Input: part model. Units: mm. Frame: model coordinates. Face numbers are marked on the shaded views. A direction names the side the tool comes from. Give positions to 0.01 mm unless a question says otherwise; leave off trailing zeros. Order: outer loops, then holes, each group sorted by start corner. A loop starts at its lowest first (then second) coordinate and runs counter-clockwise, first axis right, second up. Notation, with made-up numbers: (60.5, 57.5) - (101.5, 57.5) arc R13 cw to (101.5, 67.5) - close; hole circle Ø4 at (17, 77). An arc over 180 degrees is marked (long way). Answer in a Markdown table with one row per item. Add a question column.
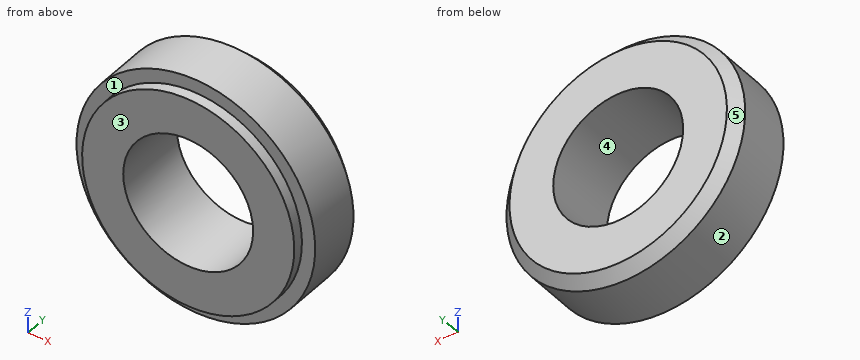
from build123d import *

# Parameters (mm, degrees)
G3_4_TAPPED_HOLE1_D     = 24.5
G3_4_TAPPED_HOLE1_DEPTH = 58.32
G3_4_TAPPED_HOLE1_TIP   = 7.360542583


with BuildPart() as part:
    # Sketch1 → Revolve1 (revolve)
    with BuildSketch(Plane(origin=(0, 0, 0), x_dir=(0, 0, -1), z_dir=(1, 0, 0))):
        Polygon((20, 0), (20, 2), (22.5, 2), (22.5, 12), (20.5, 14), (12, 14), (12, 0), align=None)
    revolve(axis=Axis((0, 0, 0), (0, 1, 0)))

    # G3/4 Tapped Hole1
    with Locations(Plane(origin=(0, 14, 0), x_dir=(1, 0, 0), z_dir=(0, 1, 0))):
        with Locations((0, 0)):
            Hole(G3_4_TAPPED_HOLE1_D / 2, depth=G3_4_TAPPED_HOLE1_DEPTH)
            with Locations((0, 0, -(G3_4_TAPPED_HOLE1_DEPTH + G3_4_TAPPED_HOLE1_TIP / 2))):  # 118° drill point
                Cone(0, G3_4_TAPPED_HOLE1_D / 2, G3_4_TAPPED_HOLE1_TIP, mode=Mode.SUBTRACT)


solid = part.part
Q1. Access query for the marked faces 1 and 2. Directions: +Z, -Z, +X, -X, +Y, -Y. A direction counts if a zero-diameter tool reaches every point of the face in a straight line with its end or side. Return the directions, or none.
Q2. Section A-A, the plane z = 0. Return loops of the section in (x, y), then the cut area to 3 significant figures.
Q3. Section C-C, the plane y = 5. Return loops of the section in (x, z), then the cut area to 3 significant figures.
Q4. Pull-direction query (X, two-part tool) for the marked faces 3, 4 and 5; classes: +X half, -X half, draft (parallel to the pull), parting line (faces both ways), or undercut.
Q5. Section B-B, the plane x = 0. Return loops of the section in (y, z).
Q6. Line query: probe 1 along Z at (x, y) = (0, 10.5); probe 2 along X at (y, z) = (2.5, 5); probe 3 along Y at (x, z) = (13, 15.5). Output: solid intervals per line, ascending.
Q7. Contact query for flat-ended pins moving along their axis: P1, Ø1.5, axis at y = 7.5, z = -3, coming from the -X side; P2, Ø1, axis at y = 2.5, z = -10.5, coming from the +X side; P3, Ø5, axis at x = 7.5, z = 2, coming from the -Y side; P4, Ø6, axis at x = 11.5, y = 5, coming from the -Z side. Output: stop coordinate, or through.
Computed:
| question | item | result |
|---|---|---|
| 1 | face 1 | -Y |
| 1 | face 2 | +Y, -Y |
| 2 | outline | (-22.5, 2) - (-20, 2) - (-20, 0) - (-12.25, 0) - (-12.25, 14) - (-20.5, 14) - (-22.5, 12) - close; (12.25, 0) - (20, 0) - (20, 2) - (22.5, 2) - (22.5, 12) - (20.5, 14) - (12.25, 14) - close |
| 2 | area | 273 mm^2 |
| 3 | outline | circle Ø45 at (0, 0); hole circle Ø24.5 at (0, 0) |
| 3 | area | 1,120 mm^2 |
| 4 | face 3 | draft |
| 4 | face 4 | undercut |
| 4 | face 5 | parting line |
| 5 | outline | (0, -20) - (2, -20) - (2, -22.5) - (12, -22.5) - (14, -20.5) - (14, -12.25) - (0, -12.25) - close; (0, 12.25) - (14, 12.25) - (14, 20.5) - (12, 22.5) - (2, 22.5) - (2, 20) - (0, 20) - close |
| 6 | probe 1 | z = -22.5 to -12.25, 12.25 to 22.5 |
| 6 | probe 2 | x = -21.94 to -11.18, 11.18 to 21.94 |
| 6 | probe 3 | y = 2 to 14 |
| 7 | P1 | stops at x = -22.39 |
| 7 | P2 | stops at x = 20.16 |
| 7 | P3 | passes through |
| 7 | P4 | stops at z = -20.83 |
